Source: three-view drawing plus pictorial views. Frame: mm from the lowest corner of the part. A direction names the side the tool comes from. Give positions to 0.01 mm unless a question says otherwise; leave off trailing zeros. Loops run counter-clockwise (first coordinate to the right, second up) from the corner with the lowest first, then second, coordinate; pieces in that order, holes last. Notation, with made-up numbers: M -29.75,60 L 23.25,60 A33 cw 23.25,94 Z; hole C 20.5,28 d1. An arc over 180 degrees is marked long. Answer as a JSON object with one key per item and string values. Group by question number.
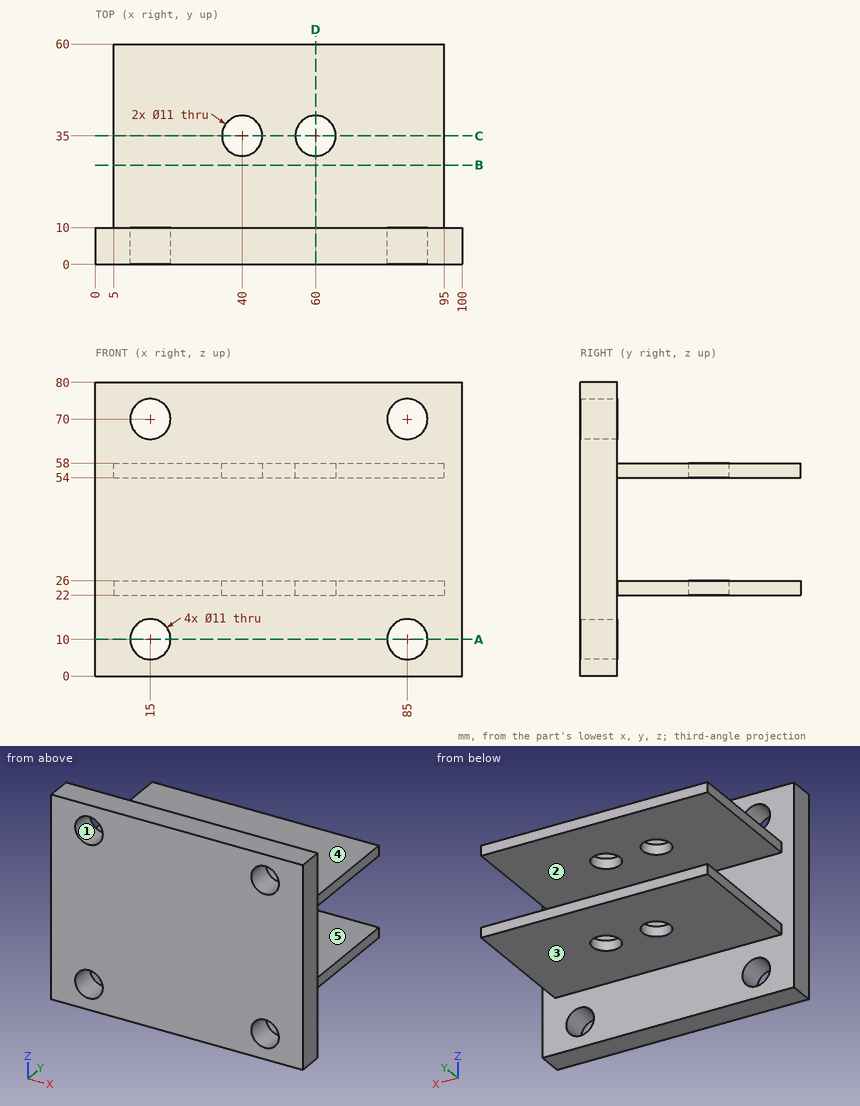
1. Material intervals for L1, parallel to Z at x = 8, y = 18; L2, parallel to Y at x = 60, z = 56.35; L3, parallel to Y at x = 53, z = 59, sorted ascending.
2. Section A-A (z = 10). Output: boundary loops of the cut face in (x, y), then the cut area to 3 significant figures.
3. First-contact query: P1, Ø15, axis at x = 33.5, y = 33, coming from the +Z side; P2, Ø9, axis at x = 40, y = 35, coming from the -Z side; P3, Ø1.2, axis at y = 42, z = 24, coming from the +X side; P4, Ø1, axis at x = 14, z = 32, coming from the +Y side. Flat tips, straight axial feed; report the tip coordinate or a pass-through.
4. Mould query, pull axis Z, two halves, no side actions, for the marked faces 3, 4 and 5. Classes: pulls with the +Z half, pulls with the -Z half, needs draft (parallel to the pull), parting line crosses it, or undercut.
5. Section C-C (y = 35). Output: boundary loops of the cut face in (x, z).
6. Section B-B (y = 27). Output: boundary loops of the cut face in (x, z), then the cut area to 3 significant figures.
7. Reachability of the marked faces 1 and 2 from +Z, -Z, +X, -X, +Y, -Y: full face, straight path, thin tool, end or side. Return the list, or none.
8. Section D-D (x = 60). Output: boundary loops of the cut face in (y, z).
Geometry results:
{
 "1": {"L1": "22 to 26, 54 to 58", "L2": "0 to 29.5, 40.5 to 60", "L3": "0 to 10"},
 "2": {"outline": "M 0,0 L 9.5,0 L 9.5,10 L 0,10 Z; M 20.5,0 L 79.5,0 L 79.5,10 L 20.5,10 Z; M 90.5,0 L 100,0 L 100,10 L 90.5,10 Z", "area": "780 mm2"},
 "3": {"P1": "z = 58", "P2": "through", "P3": "x = 95", "P4": "y = 10"},
 "4": {"face 3": "pulls with the -Z half", "face 4": "pulls with the +Z half", "face 5": "undercut"},
 "5": {"outline": "M 5,22 L 34.5,22 L 34.5,26 L 5,26 Z; M 5,54 L 34.5,54 L 34.5,58 L 5,58 Z; M 45.5,22 L 54.5,22 L 54.5,26 L 45.5,26 Z; M 45.5,54 L 54.5,54 L 54.5,58 L 45.5,58 Z; M 65.5,22 L 95,22 L 95,26 L 65.5,26 Z; M 65.5,54 L 95,54 L 95,58 L 65.5,58 Z"},
 "6": {"outline": "M 5,22 L 95,22 L 95,26 L 5,26 Z; M 5,54 L 95,54 L 95,58 L 5,58 Z", "area": "720 mm2"},
 "7": {"face 1": "+Y, -Y", "face 2": "+X, -X, +Y"},
 "8": {"outline": "M 0,0 L 10,0 L 10,22 L 29.5,22 L 29.5,26 L 10,26 L 10,54 L 29.5,54 L 29.5,58 L 10,58 L 10,80 L 0,80 Z; M 40.5,22 L 60,22 L 60,26 L 40.5,26 Z; M 40.5,54 L 60,54 L 60,58 L 40.5,58 Z"}
}
